Drawing for the job (mm, zero at the part's lowest x, y, z). Coordinates: 2 decimals unless noted, no trailing zeros. Order: outer loops, then holes, each group sorted by start corner. A loop starts at its lowest first (then second) coordinate and runs counter-clockwise, first axis right, second up. Notation, with made-up numbers: (-37, 43) - (3, 43) arc R18 cw to (3, 51) - close; hole circle Ø4 at (68.5, 9.25). An arc over 180 degrees is marked (long way). Put each result on its own line as item: value. Start each with the question number.
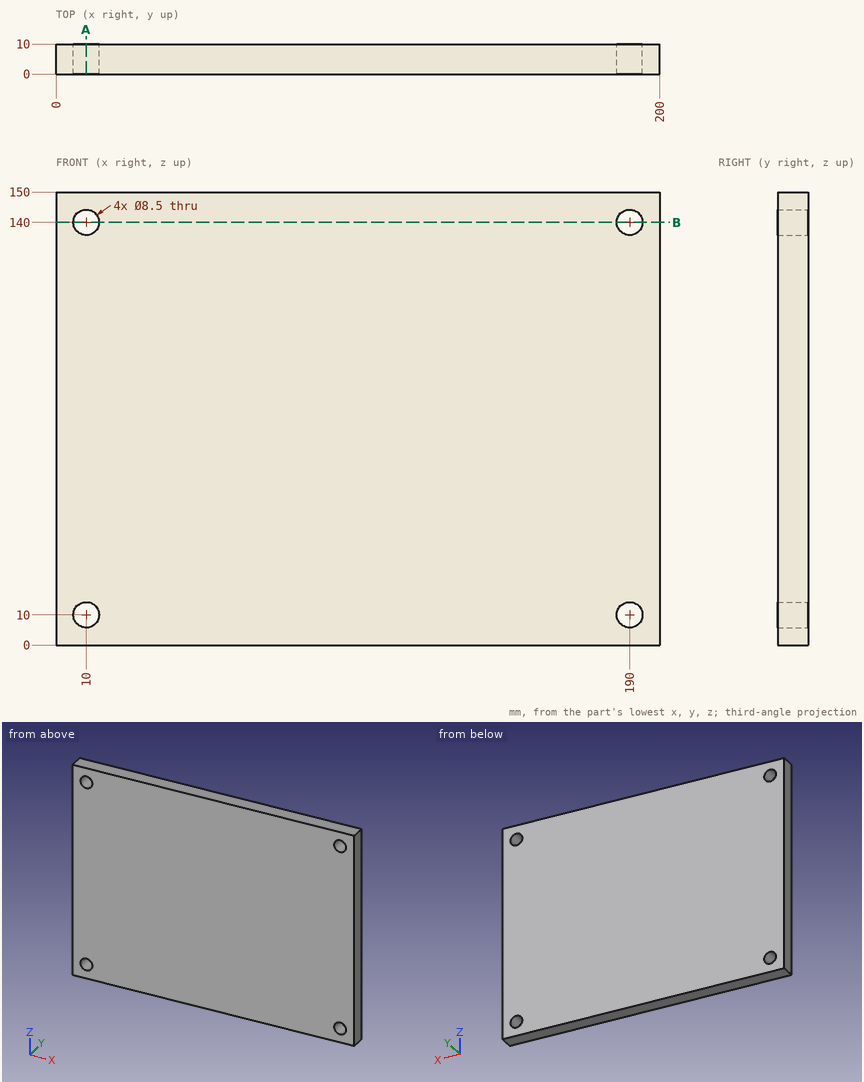
Item 1: Slice it at B-B, the plane z = 140. Give the cut face in (x, y).
Item 2: Wall check: line 1 along Z through (x, y) = (190, 6.25); line 2 along X through (y, z) = (7.25, 140); line 3 along X through (y, z) = (7.75, 11). Give the ranges that are in metal, low to high.
Item 3: Slice it at A-A, the plane x = 10. Give the cut face in (y, z).
Item 4: Flat gauge pin, fed straight in: pin 1 Ø7.5 at (x, z) = (10, 140) entering from +Y. Where does the tip first touch, or does it go through?
Here are the results:
1. outline: (0, 0) - (5.75, 0) - (5.75, 10) - (0, 10) - close; (14.25, 0) - (185.75, 0) - (185.75, 10) - (14.25, 10) - close; (194.25, 0) - (200, 0) - (200, 10) - (194.25, 10) - close
2. line 1: z = 0 to 5.75, 14.25 to 135.75, 144.25 to 150
2. line 2: x = 0 to 5.75, 14.25 to 185.75, 194.25 to 200
2. line 3: x = 0 to 5.87, 14.13 to 185.87, 194.13 to 200
3. outline: (0, 0) - (10, 0) - (10, 5.75) - (0, 5.75) - close; (0, 14.25) - (10, 14.25) - (10, 135.75) - (0, 135.75) - close; (0, 144.25) - (10, 144.25) - (10, 150) - (0, 150) - close
4. pin 1: passes through
